Verification items for this drawing (mm, ordinates from the low corner). Round coordinates to 2 decimals unless told otherwise and drop trailing zeros. Loops run counter-clockwise (first coordinate to the right, second up) from the corner with the lowest first, then second, coordinate; pieces in that order, holes last. Notation, with made-up numbers: M 4,17.5 L 55,17.5 A33 ccw 55,52.5 Z; hole C 8,-3.5 d4. An arc over 180 degrees is marked long. Write item = value, one per line. Start each with the question number.
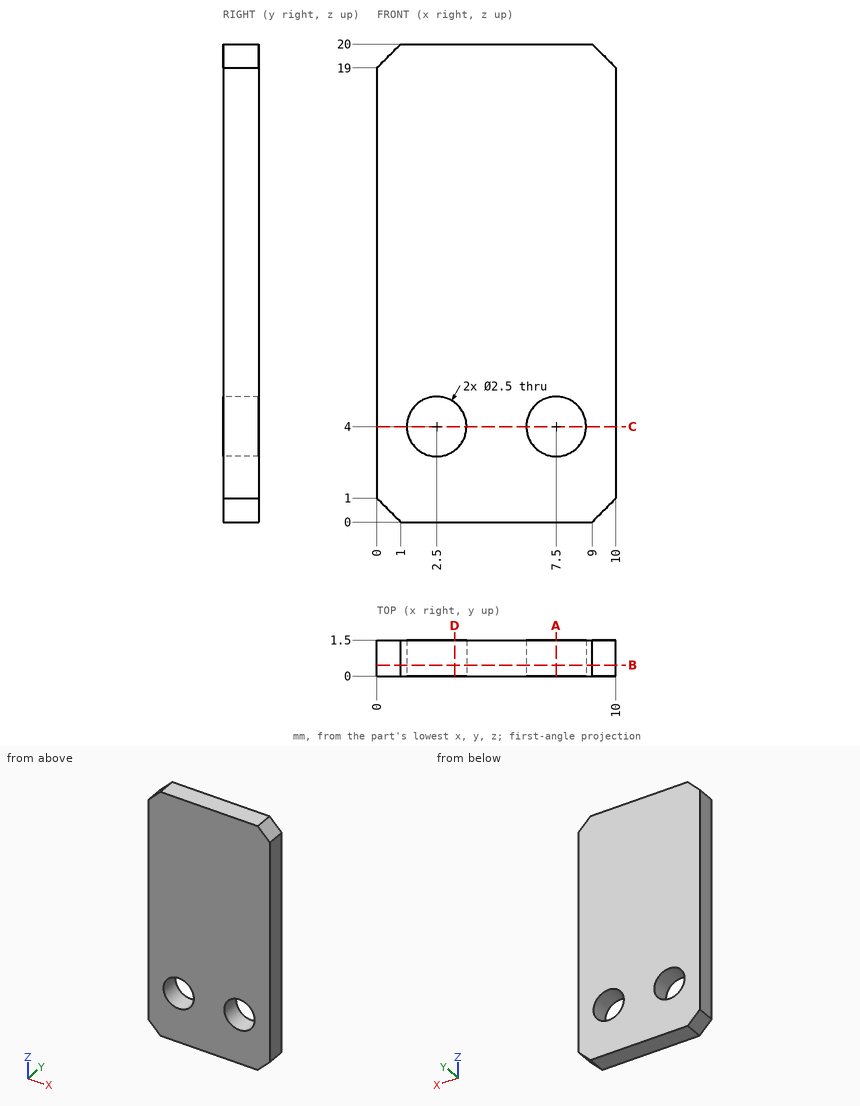
1. Section check D-D, the plane x = 3.25. Enter the section's corners in (y, z), and give its area (3 significant figures).
2. Section check A-A, the plane x = 7.5. Enter the section's corners in (y, z).
3. Thickness scan on line 1 (X direction, y = 1.15, z = 4); line 2 (X direction, y = 0.6, z = 3.5); line 3 (Z direction, x = 8.5, y = 0.85). Record the ranges inside material, lowest first.
4. Section check B-B, the plane y = 0.45. Enter the section's corners in (x, z), and give its area (3 significant figures).
5. Section check C-C, the plane z = 4. Enter the section's corners in (x, y), and give its area (3 significant figures).
Computed values:
q1.outline = M 0,0 L 1.5,0 L 1.5,3 L 0,3 Z; M 0,5 L 1.5,5 L 1.5,20 L 0,20 Z
q1.area = 27.0 mm2
q2.outline = M 0,0 L 1.5,0 L 1.5,2.75 L 0,2.75 Z; M 0,5.25 L 1.5,5.25 L 1.5,20 L 0,20 Z
q3.line_1 = 0 to 1.25, 3.75 to 6.25, 8.75 to 10
q3.line_2 = 0 to 1.35, 3.65 to 6.35, 8.65 to 10
q3.line_3 = 0 to 3.25, 4.75 to 20
q4.outline = M 0,1 L 1,0 L 9,0 L 10,1 L 10,19 L 9,20 L 1,20 L 0,19 Z; hole C 2.5,4 d2.5; hole C 7.5,4 d2.5
q4.area = 188 mm2
q5.outline = M 0,0 L 1.25,0 L 1.25,1.5 L 0,1.5 Z; M 3.75,0 L 6.25,0 L 6.25,1.5 L 3.75,1.5 Z; M 8.75,0 L 10,0 L 10,1.5 L 8.75,1.5 Z
q5.area = 7.50 mm2
